from build123d import *

# Parameters (mm, degrees)
SKETCH1_W           = 52
SKETCH1_H           = 150
BOSS_EXTRUDE1_DEPTH = 5
HOLE1_D             = 5
HOLE1_CBORE_D       = 10
HOLE1_CBORE_DEPTH   = 5


with BuildPart() as part:
    # Sketch1 → Boss-Extrude1 (new, symmetric)
    with BuildSketch(Plane.XY):
        Rectangle(SKETCH1_W, SKETCH1_H)
    extrude(amount=BOSS_EXTRUDE1_DEPTH, both=True)

    # Hole1 (through all)
    with Locations(Plane.XY.offset(5)):
        with Locations((0, 60), (0, -60), (0, 0)):
            CounterBoreHole(HOLE1_D / 2, HOLE1_CBORE_D / 2, HOLE1_CBORE_DEPTH)


solid = part.part
The listing builds one solid part. Answer for the finished solid, in the listing's coordinates (mm). A direction names the side the tool comes from. Round coordinates to 2 decimals unless told otherwise and drop trailing zeros. Loops run counter-clockwise (first coordinate to the right, second up) from the corner with the lowest first, then second, coordinate; pieces in that order, holes last. Notation, with made-up numbers: M -5,-17 L 37,-17 A31 ccw 37,7 Z; hole C 53.25,63 d6. An arc over 180 degrees is marked long. Write each question's results on one line, items separated by ' | '. Start each with the question number.
1) Which of the six approach directions +Z, -Z, +X, -X, +Y, -Y give full straight-line access (tool end or side, diameter ignored) to faces 1 (the flat face through (-6, 1, -5)), 2 (the cylindrical face through (-0.651, -55.043, 2.535))?
2) Find section C-C on x = 0. Write down the section's boundary in (y, z).
3) Each of these flat-tipped pins is pushed along its axis until it touches: pin 1 (3 mm diameter, centred on x = -0.5, y = 58.5, fed in from +Z); pin 2 (3 mm diameter, centred on x = 0, y = 0, fed in from -Z). Where does it stop, or does it pass through?
4) Straight lines are drawn through the part: probe 1 along Y at (x, z) = (0, 1.9); probe 2 along Y at (x, z) = (0, -1.55); probe 3 along X at (y, z) = (-2, -2). For each, find the intervals that lie inside material, in ascending order.
5) Find section A-A on y = 0. Write down the section's boundary in (x, z), plus the area to 3 significant figures.
6) Determine the mould class of faces 3 (the flat face through (26, -1, 0)), 4 (the cylindrical face through (-1.34, -57.89, -2.54)), 5 (the flat face through (-6, 1, 5)) for opening direction X: pulls with the +X half, pulls with the -X half, needs draft (parallel to the pull), parting line crosses it, or undercut.
7) Find section B-B on z = 2.25. Write down the section's boundary in (x, y).
Final values:
1) face 1: -Z, +X, -X, +Y, -Y | face 2: +Z
2) outline: M -75,-5 L -62.5,-5 L -62.5,0 L -65,0 L -65,5 L -75,5 Z; M -57.5,-5 L -2.5,-5 L -2.5,0 L -5,0 L -5,5 L -55,5 L -55,0 L -57.5,0 Z; M 2.5,-5 L 57.5,-5 L 57.5,0 L 55,0 L 55,5 L 5,5 L 5,0 L 2.5,0 Z; M 62.5,-5 L 75,-5 L 75,5 L 65,5 L 65,0 L 62.5,0 Z
3) pin 1: z = 0 | pin 2: through
4) probe 1: -75 to -65, -55 to -5, 5 to 55, 65 to 75 | probe 2: -75 to -62.5, -57.5 to -2.5, 2.5 to 57.5, 62.5 to 75 | probe 3: -26 to -1.5, 1.5 to 26
5) outline: M -26,-5 L -2.5,-5 L -2.5,0 L -5,0 L -5,5 L -26,5 Z; M 2.5,-5 L 26,-5 L 26,5 L 5,5 L 5,0 L 2.5,0 Z | area: 445 mm²
6) face 3: pulls with the +X half | face 4: undercut | face 5: needs draft
7) outline: M -26,-75 L 26,-75 L 26,75 L -26,75 Z; hole C 0,-60 d10; hole C 0,0 d10; hole C 0,60 d10
